from build123d import *

# Parameters (mm, degrees)
SKETCH_1_W                = 120
SKETCH_1_H                = 220
EXTRUDE_1_DEPTH           = 10
HOLE_WIZARD_2_D           = 5.5
HOLE_WIZARD_2_CBORE_D     = 9.5
HOLE_WIZARD_2_CBORE_DEPTH = 5.7
HOLE_WIZARD_3_D           = 6.6
HOLE_WIZARD_3_CBORE_D     = 11
HOLE_WIZARD_3_CBORE_DEPTH = 6.8
FILLET_1_R                = 5
CUT_EXTRUDE_1_REACH       = 127.698
SKETCH_11_W               = 120
SKETCH_11_H               = 95
HOLE_WIZARD_4_D           = 6.6
HOLE_WIZARD_4_CBORE_D     = 11
HOLE_WIZARD_4_CBORE_DEPTH = 6.8
FILLET_2_R                = 5
CUT_EXTRUDE_2_REACH       = 127.698
SKETCH_14_R               = 15
HOLE_WIZARD_5_D           = 5.5
HOLE_WIZARD_5_DEPTH       = 20.4
HOLE_WIZARD_5_CBORE_D     = 9.5
HOLE_WIZARD_5_CBORE_DEPTH = 5.7
HOLE_WIZARD_5_TIP         = 1.652366702


with BuildPart() as part:
    # 草图1 → 凸台-拉伸1 (new body)
    with BuildSketch(Plane.XY):
        Rectangle(SKETCH_1_W, SKETCH_1_H)
    extrude(amount=EXTRUDE_1_DEPTH)

    # 打孔尺寸(%根据)内六角圆柱头螺钉的类型2 (through all)
    with Locations(Plane.XY.offset(10)):
        with Locations((-55, -30), (-55, -90)):
            hole_wizard_2 = CounterBoreHole(HOLE_WIZARD_2_D / 2, HOLE_WIZARD_2_CBORE_D / 2, HOLE_WIZARD_2_CBORE_DEPTH)

    # 打孔尺寸(%根据)内六角圆柱头螺钉的类型3 (through all)
    with Locations(Plane.XY.offset(10)):
        with Locations((-20, -60), (30, -60)):
            CounterBoreHole(HOLE_WIZARD_3_D / 2, HOLE_WIZARD_3_CBORE_D / 2, HOLE_WIZARD_3_CBORE_DEPTH)

    # 圆角1
    fillet_1_edges = [part.edges().sort_by_distance(p)[0] for p in [
        (-60, 110, 5),
        (-60, -110, 5),
    ]]
    fillet(fillet_1_edges, radius=FILLET_1_R)

    # 草图11 → 切除-拉伸1 (cut, up to next)
    with BuildSketch(Plane(origin=(0, 0, 0), x_dir=(-1, 0, 0), z_dir=(0, 0, -1)), mode=Mode.PRIVATE) as cut_extrude_1_sk1:
        with Locations((0, 62.5)):
            Rectangle(SKETCH_11_W, SKETCH_11_H)
    cut_extrude_1_tool1 = extrude(cut_extrude_1_sk1.sketch, amount=-CUT_EXTRUDE_1_REACH, mode=Mode.PRIVATE) & part.part
    add(cut_extrude_1_tool1.solids().sort_by_distance((0, 62.5, 0))[0], mode=Mode.SUBTRACT)

    # 打孔尺寸(%根据)内六角圆柱头螺钉的类型4 (through all)
    with Locations(Plane(origin=(0, 0, 0), x_dir=(-1, 0, 0), z_dir=(0, 0, -1))):
        with Locations((-40, 0), (0, 0), (40, 0)):
            CounterBoreHole(HOLE_WIZARD_4_D / 2, HOLE_WIZARD_4_CBORE_D / 2, HOLE_WIZARD_4_CBORE_DEPTH)

    # 圆角2
    fillet_2_edges = [part.edges().sort_by_distance(p)[0] for p in [
        (60, 15, 5),
        (-60, 15, 5),
    ]]
    fillet(fillet_2_edges, radius=FILLET_2_R)

    # 草图14 → 切除-拉伸2 (cut, up to next)
    with BuildSketch(Plane(origin=(0, 0, 0), x_dir=(-1, 0, 0), z_dir=(0, 0, -1)), mode=Mode.PRIVATE) as cut_extrude_2_sk1:
        with Locations((-2.5, -30)):
            Circle(SKETCH_14_R)
    cut_extrude_2_tool1 = extrude(cut_extrude_2_sk1.sketch, amount=-CUT_EXTRUDE_2_REACH, mode=Mode.PRIVATE) & part.part
    # 草图14 → 切除-拉伸2 (cut, up to next)
    with BuildSketch(Plane(origin=(0, 0, 0), x_dir=(-1, 0, 0), z_dir=(0, 0, -1)), mode=Mode.PRIVATE) as cut_extrude_2_sk2:
        with Locations((-2.5, -80)):
            Circle(SKETCH_14_R)
    cut_extrude_2_tool2 = extrude(cut_extrude_2_sk2.sketch, amount=-CUT_EXTRUDE_2_REACH, mode=Mode.PRIVATE) & part.part
    add(cut_extrude_2_tool1.solids().sort_by_distance((2.5, -30, 0))[0], mode=Mode.SUBTRACT)
    add(cut_extrude_2_tool2.solids().sort_by_distance((2.5, -80, 0))[0], mode=Mode.SUBTRACT)

    # 镜向1: 打孔尺寸(%根据)内六角圆柱头螺钉的类型2 across plane
    add(hole_wizard_2.mirror(Plane(origin=(0, 0, 0), x_dir=(0, 0, 1), z_dir=(1, 0, 0))), mode=Mode.SUBTRACT)

    # 打孔尺寸(%根据)内六角圆柱头螺钉的类型5
    with Locations(Plane.XY.offset(10)):
        with Locations((20, -105), (-30, -105)):
            CounterBoreHole(HOLE_WIZARD_5_D / 2, HOLE_WIZARD_5_CBORE_D / 2, HOLE_WIZARD_5_CBORE_DEPTH, depth=HOLE_WIZARD_5_DEPTH)
            with Locations((0, 0, -(HOLE_WIZARD_5_DEPTH + HOLE_WIZARD_5_TIP / 2))):  # 118° drill point
                Cone(0, HOLE_WIZARD_5_D / 2, HOLE_WIZARD_5_TIP, mode=Mode.SUBTRACT)


solid = part.part
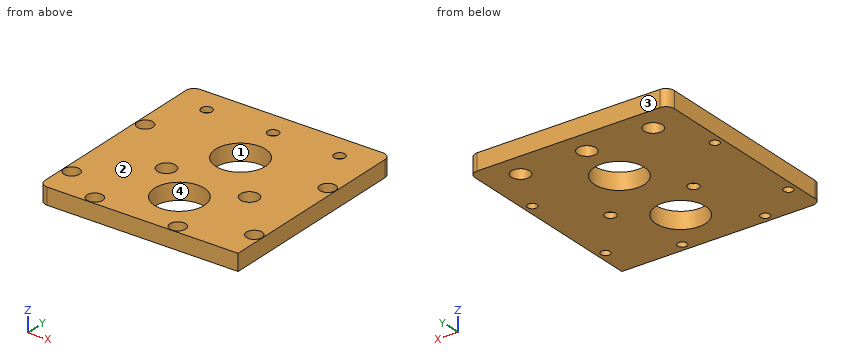
Design review of the part built by this model. Coordinates are the model's own, in mm. Face numbers are marked on the shaded views. Round coordinates to 2 decimals unless told otherwise and drop trailing zeros. Write each loop counter-clockwise with the first axis right and the second up, starting at its lowest first coordinate (ties: lowest second). Pieces come first, ordered by that corner, then holes. Notation, with made-up numbers: (34.25, 1.5) - (63.25, 1.5) arc R12 cw to (63.25, 15.5) - close; hole circle Ø2 at (-12, 44.25). An arc over 180 degrees is marked (long way). Use a Markdown table: item, result. Add a question column.
1. Clearance check with flat-ended pins moving along their axes: pin 1 (7 mm diameter, centred on x = -30, y = -105, fed in from +Z); pin 2 (3.5 mm diameter, centred on x = -41.5, y = -2, fed in from -Z); pin 3 (6.5 mm diameter, centred on x = -55, y = -30, fed in from -Z); pin 4 (6 mm diameter, centred on x = 30, y = -60, fed in from -Z). State where each tip first meets the part, or that it passes through.
2. Mouldability with a two-part tool opening along Y and no side actions: class the marked faces 1, 2, 3 and 4 as +Y half, -Y half, draft (parallel to the pull), parting line (faces both ways), or undercut.
3. We need section A-A (y = -80). State the section outline as (x, z) points, then the cut area to 3 significant figures.
4. We need section D-D (y = -39). State the section outline as (x, z) points.
5. We need section B-B (x = 20). State the section outline as (y, z) points, then the cut area to 3 significant figures.
6. We need section C-C (x = -10.5). State the section outline as (y, z) points, then the cut area to 3 significant figures.
7. Wall thickness on probe 1 along Y at (x, z) = (-55, 1.75); probe 2 along Y at (x, z) = (-55, 7); probe 3 along Y at (x, z) = (30, 3): over which ranges is each line inside the solid? List them lowest first.
Output:
| question | item | result |
|---|---|---|
| 1 | pin 1 | stops at z = 4.3 |
| 1 | pin 2 | stops at z = 6.8 |
| 1 | pin 3 | stops at z = 0 |
| 1 | pin 4 | passes through |
| 2 | face 1 | undercut |
| 2 | face 2 | draft |
| 2 | face 3 | +Y half |
| 2 | face 4 | undercut |
| 3 | outline | (-60, 0) - (-12.5, 0) - (-12.5, 10) - (-60, 10) - close; (17.5, 0) - (60, 0) - (60, 10) - (17.5, 10) - close |
| 3 | area | 900 mm2 |
| 4 | outline | (-60, 0) - (-9.5, 0) - (-9.5, 10) - (-60, 10) - close; (14.5, 0) - (60, 0) - (60, 10) - (14.5, 10) - close |
| 5 | outline | (-110, 0) - (-107.75, 0) - (-107.75, 4.3) - (-109.75, 4.3) - (-109.75, 10) - (-110, 10) - close; (-102.25, 0) - (15, 0) - (15, 10) - (-100.25, 10) - (-100.25, 4.3) - (-102.25, 4.3) - close |
| 5 | area | 1,170 mm2 |
| 6 | outline | (-110, 0) - (-87.48, 0) - (-87.48, 10) - (-110, 10) - close; (-72.52, 0) - (-37.48, 0) - (-37.48, 10) - (-72.52, 10) - close; (-22.52, 0) - (15, 0) - (15, 10) - (-22.52, 10) - close |
| 6 | area | 951 mm2 |
| 7 | probe 1 | y = -110 to -92.75, -87.25 to -32.75, -27.25 to 15 |
| 7 | probe 2 | y = -110 to -94.75, -85.25 to -34.75, -25.25 to 15 |
| 7 | probe 3 | y = -110 to -63.3, -56.7 to 15 |
